Part model, mm, in its own coordinate system. Face numbers are marked on the shaded views. A direction names the side the tool comes from. Give positions to 0.01 mm unless a question says otherwise; leave off trailing zeros. Write each loop counter-clockwise with the first axis right and the second up, starting at its lowest first coordinate (ties: lowest second). Pieces come first, ordered by that corner, then holes. Notation, with made-up numbers: M -32,-23 L -18,-23 A32 ccw -18,4 Z; hole C -37.5,9.25 d1. An arc over 180 degrees is marked long. Answer as CSV lines item,"result". Start each with the question number.
Item 1: Two-plate mould, pull along Z, no slides. Class the marked faces 1 and 2: +Z half, -Z half, draft (parallel to the pull), parting line (faces both ways), or undercut.
Item 2: Pin check, flat tips, straight feed: pin 1 (2 mm diameter, centred on x = 5.5, z = -1.5, fed in from +Y); pin 2 (0.9 mm diameter, centred on y = 0, z = -0.5, fed in from -X); pin 3 (2 mm diameter, centred on x = 7.5, z = -0.5, fed in from +Y). Stop position of each tip, or through.
Item 3: Wall check: L1, parallel to X at y = 0.25, z = 0.8; L2, parallel to X at y = -1.5, z = 0.9; L3, parallel to Y at x = 6, z = -0.55. Give the ranges that are in metal, low to high. Write a range as from..to.
Item 4: Band-saw the part on C-C, the plane x = 2.5. List the corners of the cut face in (y, z).
Item 5: 3-axis set-ups, long thin cutter, end or side, ignore diameter. For the marked faces 3 and 4: which of +Z, -Z, +X, -X, +Y, -Y reach the whole face in a straight line?
Item 6: Band-saw the part on D-D, the plane x = 1. List the corners of the cut face in (y, z), then the cut area to 3 significant figures.
Item 7: Band-saw the part on B-B, the plane y = 0. List the corners of the cut face in (x, z), then the cut area to 3 significant figures.
Item 8: Band-saw the part on A-A, the plane z = 0. List the corners of the cut face in (x, y).
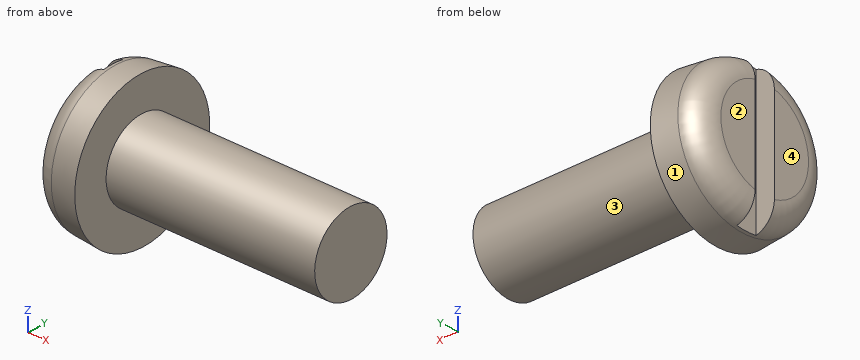
from build123d import *

# Parameters (mm, degrees)
FILLET2_R  = 0.9
SKETCH2_W  = 5.6
SKETCH2_H  = 0.8
SLOT_DEPTH = 0.7


with BuildPart() as part:
    # BodySke → Base-Revolve (revolve)
    with BuildSketch(Plane.XY, mode=Mode.PRIVATE) as base_revolve_sk:
        Polygon((1.8, 1.5), (1.8, 2.8), (0, 2.642520406), (0, 0), (9.8, 0), (9.8, 1.5), align=None)
    revolve(base_revolve_sk.sketch.rotate(Axis((-25.4, 0, 0), (1, 0, 0)), 90), axis=Axis((-25.4, 0, 0), (1, 0, 0)))

    # Fillet2
    fillet2_edges = [part.edges().sort_by_distance(p)[0] for p in [
        (0, 0, -2.642520406),
    ]]
    fillet(fillet2_edges, radius=FILLET2_R)

    # Sketch2 → Slot (cut)
    with BuildSketch(Plane(origin=(0, 0, 0), x_dir=(0, 0, -1), z_dir=(1, 0, 0))):
        Rectangle(SKETCH2_W, SKETCH2_H)
    extrude(amount=SLOT_DEPTH, mode=Mode.SUBTRACT)


solid = part.part
Output:
1,face 1,"parting line"
1,face 2,"draft"
2,pin 1,"y = 1.41"
2,pin 2,"x = 0"
2,pin 3,"y = 1.5"
3,L1,"0.7..9.8"
3,L2,"0..1.8"
3,L3,"-1.4..1.4"
4,outline,"C 0,0 d3"
5,face 3,"+X"
5,face 4,"+Z, -Z, -X, +Y, -Y"
6,outline,"C 0,0 d5.46"
6,area,"23.4 mm²"
7,outline,"M 0.7,-2.7 A0.9 ccw 0.82,-2.71 L 1.8,-2.8 L 1.8,-1.5 L 9.8,-1.5 L 9.8,1.5 L 1.8,1.5 L 1.8,2.8 L 0.82,2.71 A0.9 ccw 0.7,2.7 Z"
7,area,"30.1 mm²"
8,outline,"M 0,-1.82 A0.9 ccw 0.82,-2.71 L 1.8,-2.8 L 1.8,-1.5 L 9.8,-1.5 L 9.8,1.5 L 1.8,1.5 L 1.8,2.8 L 0.82,2.71 A0.9 ccw 0,1.82 L 0,0.4 L 0.7,0.4 L 0.7,-0.4 L 0,-0.4 Z"
